Can you work these out from the model? Positions are in its coordinate system, mm. A direction names the side the tool comes from. Round coordinates to 2 decimals unless told otherwise and drop trailing zeros. Order: outer loops, then holes, each group sorted by start corner. A loop starts at its lowest first (then second) coordinate and runs counter-clockwise, first axis right, second up. Notation, with made-up numbers: (1, 33.5) - (32, 33.5) arc R31 ccw to (32, 59.5) - close; hole circle Ø4 at (73, -37.5). An arc over 180 degrees is marked (long way). Write item = value, one per line.
from build123d import *

# Parameters (mm, degrees)
SKETCH1_R                   = 6
BOSS_EXTRUDE1_DEPTH         = 170
CHAMFER1_SIZE               = 1
CUT_EXTRUDE1_DEPTH          = 171.211632975
CUT_EXTRUDE1_DEPTH_BACK     = 171.211632975
SKETCH2_W                   = 2
SKETCH2_H                   = 50
M4_TAPPED_HOLE1_D           = 3.3
M4_TAPPED_HOLE1_CSINK_D     = 4.05
M4_TAPPED_HOLE1_CSINK_ANGLE = 90


with BuildPart() as part:
    # Sketch1 → Boss-Extrude1 (new body)
    with BuildSketch(Plane.XY):
        Circle(SKETCH1_R)
    extrude(amount=BOSS_EXTRUDE1_DEPTH)

    # Chamfer1
    chamfer1_edges = [part.edges().sort_by_distance(p)[0] for p in [
        (-6, 0, 0),
        (-6, 0, 170),
    ]]
    chamfer(chamfer1_edges, length=CHAMFER1_SIZE)

    # Sketch2 → Cut-Extrude1 (cut, two sides: drawn at the far end of the back side and taken through both)
    with BuildSketch(Plane(origin=(0, 0, 0), x_dir=(1, 0, 0), z_dir=(0, 1, 0)).offset(-CUT_EXTRUDE1_DEPTH_BACK)):
        with Locations((-5, -145)):
            Rectangle(SKETCH2_W, SKETCH2_H)
        with Locations((5, -145)):
            Rectangle(SKETCH2_W, SKETCH2_H)
    extrude(amount=CUT_EXTRUDE1_DEPTH + CUT_EXTRUDE1_DEPTH_BACK, mode=Mode.SUBTRACT)

    # M4 Tapped Hole1 (through all)
    with Locations(Plane.ZY.offset(4)):
        with Locations((160, 0), (145, 0)):
            CounterSinkHole(M4_TAPPED_HOLE1_D / 2, M4_TAPPED_HOLE1_CSINK_D / 2, counter_sink_angle=M4_TAPPED_HOLE1_CSINK_ANGLE)


solid = part.part
(1) Thinking about a two-plate mould opening in Z: for faces 1 (the face through (-4, -3, 145)), 2 (the face through (0.1, 5.2, 169.8)), 3 (the face through (0.241, 0.496, 143.426)), which applies, +Z half, -Z half, draft (parallel to the pull), parting line (faces both ways), or undercut?
Computed:
face_1 = draft
face_2 = +Z half
face_3 = undercut
(2) On a 3-axis mill with a long thin cutter (end or side, diameter ignored), from which of +Z, -Z, +X, -X, +Y, -Y can I reach the whole of each face in a straight line? I mean faces 4 (the face through (0, 0, 0)), 5 (the face through (4, -2, 145)). Say none if no direction works.
Computed:
face_4 = -Z, +X, -X, +Y, -Y
face_5 = +Z, +X, +Y, -Y
(3) If we section it at B-B (y = 0): Write out the boundary of the cut face in (x, z) (3 decimals), plus the area to 3 significant figures.
Computed:
outline = (-6, 1) - (-5, 0) - (5, 0) - (6, 1) - (6, 120) - (4, 120) - (4, 143.35) - (-3.625, 143.35) - (-4, 142.975) - (-4, 120) - (-6, 120) - close; (-4, 147.025) - (-3.625, 146.65) - (4, 146.65) - (4, 158.35) - (-3.625, 158.35) - (-4, 157.975) - close; (-4, 162.025) - (-3.625, 161.65) - (4, 161.65) - (4, 170) - (-4, 170) - close
area = 1,790 mm^2
(4) If we section it at D-D (z = 25): Write out the boundary of the cut face in (x, y), plus the area to 3 significant figures.
Computed:
outline = circle Ø12 at (0, 0)
area = 113 mm^2
(5) Will these pins go through, and if not, where does the flat tip stop? P1, Ø5, axis at x = -4, z = 47, coming from the +Y side; P2, Ø2.5, axis at y = 0, z = 160, coming from the -X side; P3, Ø1.6, axis at x = -5, y = 2, coming from the +Z side; P4, Ø1.5, axis at x = -4, z = 125, coming from the +Y side.
Computed:
P1 = 5.81
P2 = through
P3 = 120
P4 = 5.04
(6) If I drill on line 1 (Z direction, x = 1, y = 0); line 2 (Y direction, x = 0.25, z = 160); line 3 (Z direction, x = 1.75, y = 1.5), over which ranges is the centre line in solid material (lowest first)? Write a range as from..to.
Computed:
line_1 = 0..143.35, 146.65..158.35, 161.65..170
line_2 = -5.99..-1.65, 1.65..5.99
line_3 = 0..144.31, 145.69..159.31, 160.69..170
(7) If we section it at A-A (z = 145): Write out the boundary of the cut face in (x, y) (3 decimals).
Computed:
outline = (-4, -4.472) arc R6 ccw to (4, -4.472) - (4, -1.65) - (-3.625, -1.65) - (-4, -2.025) - close; (-4, 2.025) - (-3.625, 1.65) - (4, 1.65) - (4, 4.472) arc R6 ccw to (-4, 4.472) - close
(8) If we section it at C-C (x = -2.25): State how many separate pieces and enclosed holes the cut face has, plus the area to 3 significant figures.
Computed:
separate_pieces = 1
enclosed_holes = 2
area = 1,870 mm^2
